```python
from build123d import *

# Parameters (mm, degrees)
SKETCH1_W            = 40
SKETCH1_H            = 40
BOSS_EXTRUDE1_DEPTH  = 40
CUT_EXTRUDE1_DEPTH   = 40
SKETCH3_W            = 36
SKETCH3_H            = 32
CUT_EXTRUDE2_DEPTH   = 36
SKETCH4_W            = 36
SKETCH4_H            = 6
SKETCH4_W_2          = 29
SKETCH4_H_2          = 10
CUT_EXTRUDE3_DEPTH   = 2.6
BOSS_EXTRUDE2_DEPTH  = 10
SKETCH6_W            = 35.3
SKETCH6_H            = 1.25
CUT_EXTRUDE4_DEPTH   = 10
BOSS_EXTRUDE3_DEPTH  = 6
LPATTERN1_COUNT      = 2
LPATTERN1_PITCH      = 28.4
CUT_EXTRUDE5_DEPTH   = 5
MIRROR1_COPY_1_DEPTH = 6
FILLET1_R            = 1


with BuildPart() as part:
    # Sketch1 → Boss-Extrude1 (new body)
    with BuildSketch(Plane.XY):
        with Locations((-20, 20)):
            Rectangle(SKETCH1_W, SKETCH1_H)
    extrude(amount=BOSS_EXTRUDE1_DEPTH)

    # Sketch2 → Cut-Extrude1 (cut)
    with BuildSketch(Plane.XY.offset(40)):
        Polygon((-32, 40), (-32, 33.5), (-6.610595609, 8), (0, 8), (17.085067255, 36.265731876), (-7.495565519, 45.713912599), align=None)
    extrude(amount=-CUT_EXTRUDE1_DEPTH, mode=Mode.SUBTRACT)

    # Sketch3 → Cut-Extrude2 (cut)
    with BuildSketch(Plane(origin=(0, 40, 0), x_dir=(1, 0, 0), z_dir=(0, 1, 0))):
        with Locations((-18, -20)):
            Rectangle(SKETCH3_W, SKETCH3_H)
    extrude(amount=-CUT_EXTRUDE2_DEPTH, mode=Mode.SUBTRACT)

    # Sketch4 → Cut-Extrude3 (cut)
    with BuildSketch(Plane.XZ):
        with Locations((-19.8, 34.2)):
            Rectangle(SKETCH4_W, SKETCH4_H)
        with Locations((-20.5, 20)):
            Rectangle(SKETCH4_W_2, SKETCH4_H_2)
        with Locations((-19.8, 5.8)):
            Rectangle(SKETCH4_W, SKETCH4_H)
    cut_extrude3 = extrude(amount=-CUT_EXTRUDE3_DEPTH, mode=Mode.SUBTRACT)

    # Sketch5 → Boss-Extrude2 (add)
    with BuildSketch(Plane(origin=(0, 0, 25), x_dir=(-1, 0, 0), z_dir=(0, 0, -1))):
        Polygon((31.8, 2.6), (35, 2.6), (38, 2.6), (38, -2.5), align=None)
        Polygon((6, 0), (6, -2.5), (2.7, 0), align=None)
    boss_extrude2 = extrude(amount=BOSS_EXTRUDE2_DEPTH)

    # Sketch6 → Cut-Extrude4 (cut)
    with BuildSketch(Plane.XZ):
        with Locations((-20.35, 15.625)):
            Rectangle(SKETCH6_W, SKETCH6_H)
        with Locations((-20.35, 24.375)):
            Rectangle(SKETCH6_W, SKETCH6_H)
    cut_extrude4 = extrude(amount=CUT_EXTRUDE4_DEPTH, mode=Mode.SUBTRACT)

    # Sketch7 → Boss-Extrude3 (add)
    with BuildSketch(Plane(origin=(0, 0, 8.8), x_dir=(-1, 0, 0), z_dir=(0, 0, -1))):
        Polygon((37.8, 0), (34.3, 2.6), (37.8, 2.6), align=None)
    boss_extrude3 = extrude(amount=BOSS_EXTRUDE3_DEPTH)

    # LPattern1: Boss-Extrude3 ×2
    with Locations(*[(0, 0, i * LPATTERN1_PITCH) for i in range(1, LPATTERN1_COUNT)]):
        add(boss_extrude3)

    # Sketch9 → Cut-Extrude5 (cut)
    with BuildSketch(Plane.XZ.offset(-2.6)):
        with BuildLine():
            Line((-27.3, 24.5), (-12.7, 24.5))
            ThreePointArc((-12.7, 24.5), (-8.2, 20), (-12.7, 15.5))
            Line((-12.7, 15.5), (-27.3, 15.5))
            ThreePointArc((-27.3, 15.5), (-31.8, 20), (-27.3, 24.5))
        make_face()
    cut_extrude5 = extrude(amount=-CUT_EXTRUDE5_DEPTH, mode=Mode.SUBTRACT)

    # Mirror1: Cut-Extrude3, Boss-Extrude2, Cut-Extrude4, Boss-Extrude3, Cut-Extrude5 across plane
    add(cut_extrude3.mirror(Plane(origin=(-20, 20, 0), x_dir=(0, 0, 1), z_dir=(-0.7071067811865475, 0.7071067811865477, 0))), mode=Mode.SUBTRACT)
    add(boss_extrude2.mirror(Plane(origin=(-20, 20, 0), x_dir=(0, 0, 1), z_dir=(-0.7071067811865475, 0.7071067811865477, 0))))
    add(cut_extrude4.mirror(Plane(origin=(-20, 20, 0), x_dir=(0, 0, 1), z_dir=(-0.7071067811865475, 0.7071067811865477, 0))), mode=Mode.SUBTRACT)
    add(boss_extrude3.mirror(Plane(origin=(-20, 20, 0), x_dir=(0, 0, 1), z_dir=(-0.7071067811865475, 0.7071067811865477, 0))))
    add(cut_extrude5.mirror(Plane(origin=(-20, 20, 0), x_dir=(0, 0, 1), z_dir=(-0.7071067811865475, 0.7071067811865477, 0))), mode=Mode.SUBTRACT)

    # Mirror1 copy 1 sketch → Mirror1 copy 1 (add)
    with BuildSketch(Plane(origin=(-40, 40, 37.2), x_dir=(0, -1, 0), z_dir=(0, 0, -1))):
        Polygon((37.8, 0), (34.3, -2.6), (37.8, -2.6), align=None)
    extrude(amount=MIRROR1_COPY_1_DEPTH)

    # Fillet1
    fillet1_edges = [part.edges().sort_by_distance(p)[0] for p in [
        (-32, 40, 2),
        (0, 8, 2),
        (-32, 40, 38),
        (0, 8, 38),
        (-40, 0, 20),
    ]]
    fillet(fillet1_edges, radius=FILLET1_R)


solid = part.part
```
CAD build for the part. Positions are in the model's coordinates, mm. A direction names the side the tool comes from. Give positions to 0.01 mm unless a question says otherwise; leave off trailing zeros. Write each loop counter-clockwise with the first axis right and the second up, starting at its lowest first coordinate (ties: lowest second). Pieces come first, ordered by that corner, then holes. Notation, with made-up numbers: (54.5, 48) -> (84.5, 48) arc R24 ccw to (84.5, 69) -> close; hole circle Ø10 at (-11, -17). An arc over 180 degrees is marked (long way). Write each question's results on one line, items separated by ' | '.
1. Two-plate mould, pull along X, no slides. Class faces 6 (the flat face through (-20, 3, 15.5)), 7 (the flat face through (-37.4, 22, 6)), 8 (the flat face through (-37, -1, 23.75)): pulls with the +X half, pulls with the -X half, needs draft (parallel to the pull), parting line crosses it, or undercut.
Geometry check:
face 6: undercut | face 7: pulls with the -X half | face 8: needs draft
2. Cut at B-B, the plane y = 23. Write the cut outline in (x, z).
Geometry check:
outline: (-40, 0) -> (-21.55, 0) -> (-21.55, 4) -> (-36, 4) -> (-36, 15.5) -> (-37.4, 15.5) -> (-37.4, 15) -> (-40, 15) -> (-40, 8.8) -> (-37.4, 8.8) -> (-37.4, 2.8) -> (-40, 2.8) -> close; (-40, 25) -> (-37.4, 25) -> (-37.4, 24.5) -> (-36, 24.5) -> (-36, 36) -> (-21.55, 36) -> (-21.55, 40) -> (-40, 40) -> (-40, 37.2) -> (-37.4, 37.2) -> (-37.4, 31.2) -> (-40, 31.2) -> close
3. Wall check: probe 1 along Z at (x, y) = (-38, 34.5); probe 2 along Z at (x, y) = (-29, 5); probe 3 along X at (y, z) = (5, 26). Give the ranges that are in metal, low to high. Write a range as [from, to].
Geometry check:
probe 1: [0, 2.8], [8.8, 31.2], [37.2, 40] | probe 2: [0, 4], [36, 40] | probe 3: [-40, -36]
4. Which spindle directions (+Z, -Z, +X, -X, +Y, -Y) get a long thin tool onto all of the face, cutting with end or side? Do faces 1 (the flat face through (-38.718, 3.926, 34.242)), 2 (the flat face through (-37, -1, 16.25)), 3 (the flat face through (-32, 36, 2)), 4 (the flat face through (-20, 3, 24.5)), 5 (the flat face through (-38, -1, 20)). Say none if no direction does.
Geometry check:
face 1: -X | face 2: -Z, +X, -X, -Y | face 3: +Z, -Z, +X, +Y | face 4: +Y, -Y | face 5: +Z, -Z, -X, -Y
5. Drop flat-ended pins along their axis: P1, Ø1.3, axis at x = -41.5, y = 4, coming from the -Z side; P2, Ø5, axis at y = 35.5, z = 35, coming from the -X side; P3, Ø12, axis at x = -22, z = 18.5, coming from the +Y side. Give the stop position or say it passes through.
Geometry check:
P1: z = 16.25 | P2: x = -40 | P3: y = 4
6. Cut at C-C, the plane x = -28. Write the cut outline in (y, z).
Geometry check:
outline: (0, 0) -> (29.48, 0) -> (29.48, 4) -> (4, 4) -> (4, 15.55) -> (2.6, 15.55) -> (2.6, 15) -> (0, 15) -> (0, 8.8) -> (2.6, 8.8) -> (2.6, 2.8) -> (0, 2.8) -> close; (0, 25) -> (2.6, 25) -> (2.6, 24.45) -> (4, 24.45) -> (4, 36) -> (29.48, 36) -> (29.48, 40) -> (0, 40) -> (0, 37.2) -> (2.6, 37.2) -> (2.6, 31.2) -> (0, 31.2) -> close
7. Cut at A-A, the plane z = 28.5. Write the cut outline in (x, y), then the cut area to 3 significant figures.
Geometry check:
outline: (-40, 1) arc R1 ccw to (-39, 0) -> (0, 0) -> (0, 4) -> (-36, 4) -> (-36, 40) -> (-40, 40) -> close | area: 304 mm²
8. Cut at D-D, the plane z = 7.5. Write the cut outline in (x, y).
Geometry check:
outline: (-40, 1) arc R1 ccw to (-39, 0) -> (-37.8, 0) -> (-34.3, 2.6) -> (-1.8, 2.6) -> (-1.8, 0) -> (0, 0) -> (0, 4) -> (-36, 4) -> (-36, 40) -> (-40, 40) -> (-40, 38.2) -> (-37.4, 38.2) -> (-37.4, 5.7) -> (-40, 2.2) -> close
